from build123d import *

# Parameters (mm, degrees)
BOSS_EXTRUDE1_DEPTH = 9
SKETCH2_R           = 15
BOSS_EXTRUDE2_DEPTH = 4
SKETCH3_R           = 7.5
BOSS_EXTRUDE3_DEPTH = 2
SKETCH4_R           = 11
BOSS_EXTRUDE5_DEPTH = 13
CHAMFER1_SIZE       = 2
SCALE_1_SCALE       = 1.875


with BuildPart() as part:
    # Sketch1 → Boss-Extrude1 (new body)
    with BuildSketch(Plane.XY):
        Polygon((14.43375673, 0), (7.216878365, 12.5), (-7.216878365, 12.5), (-14.43375673, 0), (-7.216878365, -12.5), (7.216878365, -12.5), align=None)
    extrude(amount=BOSS_EXTRUDE1_DEPTH)

    # Sketch2 → Boss-Extrude2 (add)
    with BuildSketch(Plane.XY.offset(9)):
        Circle(SKETCH2_R)
    extrude(amount=BOSS_EXTRUDE2_DEPTH)

    # Sketch3 → Boss-Extrude3 (add)
    with BuildSketch(Plane.XY.offset(13)):
        Circle(SKETCH3_R)
    extrude(amount=BOSS_EXTRUDE3_DEPTH)

    # Sketch4 → Boss-Extrude5 (add)
    with BuildSketch(Plane.XY.offset(15)):
        with Locations(Location((0, 0, 0), (0, 0, 180))):
            Circle(SKETCH4_R)
    extrude(amount=BOSS_EXTRUDE5_DEPTH)

    # Chamfer1
    chamfer1_edges = [part.edges().sort_by_distance(p)[0] for p in [
        (11, 0, 28),
    ]]
    chamfer(chamfer1_edges, length=CHAMFER1_SIZE)

    # Sketch6 → Cut-Revolve4 (revolve, cut)
    with BuildSketch(Plane(origin=(0, 0, 0), x_dir=(1, 0, 0), z_dir=(0, 1, 0)), mode=Mode.PRIVATE) as cut_revolve4_sk:
        with BuildLine():
            Line((-10.43375673, 0), (-11.300713231, 3.45481125))
            Line((-11.300713231, 3.45481125), (-14.43375673, 0))
            Line((-14.43375673, 0), (-14.43375673, -1))
            ThreePointArc((-14.43375673, -1), (-12.499286844, -0.237879543), (-10.43375673, 0))
        make_face()
    revolve(cut_revolve4_sk.sketch.rotate(Axis((0, 0, 0), (0, 0, -1)), 180), axis=Axis((0, 0, 0), (0, 0, -1)), mode=Mode.SUBTRACT)


with BuildPart() as part_1:
    # Scale 1: scaled about (-3.1e-08, 2.41e-07, 12.521211358)
    add(part.part.scale(SCALE_1_SCALE).moved(Location((2.7e-08, -2.11e-07, -10.956059938))))


solid = part_1.part
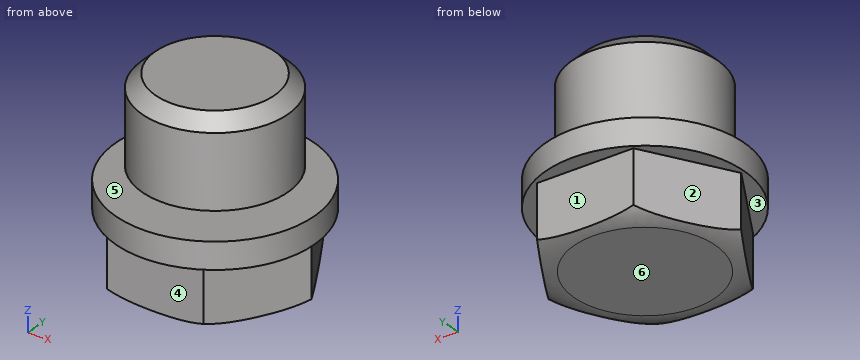
Design review of the part built by this model. Coordinates are the model's own, in mm. Face numbers are marked on the shaded views. A direction names the side the tool comes from. Round coordinates to 2 decimals unless told otherwise and drop trailing zeros. Write each loop counter-clockwise with the first axis right and the second up, starting at its lowest first coordinate (ties: lowest second). Pieces come first, ordered by that corner, then holes. Notation, with made-up numbers: M 35.25,-14 L 45.25,-14 A38 cw 45.25,25 Z; hole C 5,68.25 d4. An arc over 180 degrees is marked long. One line per item, written item: value. Start each with the question number.
1. To check wall thickness, follow probe 1 along Z at (x, y) = (13, -19.5); probe 2 along Y at (x, z) = (-9, -8.5); probe 3 along Z at (x, y) = (11, -13). State the ranges of each line that lie inside material, in increasing order. Write a range as from..to.
2. Draft analysis for pull direction Z (two halves, no side actions). For the marked faces 4, 5 and 6, state which applies: pulls with the +Z half, pulls with the -Z half, needs draft (parallel to the pull), parting line crosses it, or undercut.
3. Take a section at B-B on z = 25.5. State the section outline as (x, y) points (3 decimals).
4. Clearance check with flat-ended pins moving along their axes: P1, Ø8, axis at x = 6, z = 32.5, coming from the -Y side; P2, Ø13, axis at x = 5, z = -1.5, coming from the +Y side; P3, Ø1.5, axis at x = 0, z = 30, coming from the -Y side (3 decimals). State where each tip first meets the part, or that it passes through.
5. Take a section at C-C on z = 9.5. State the section outline as (x, y) points (3 decimals), then the cut area to 3 significant figures.
6. Take a section at A-A on z = 0.5. State the section outline as (x, y) points.
7. For the marked faces 1, 2 and 3, list the 3-axis set-ups (+Z, -Z, +X, -X, +Y, -Y) from which the entire face can be reached by the end or side of a thin tool; tool diameter is ignored.
Computed:
1. probe 1: z = -10.51..13.42
1. probe 2: y = -23.44..23.44
1. probe 3: z = -10.96..13.42, 17.17..41.39
2. face 4: needs draft
2. face 5: undercut
2. face 6: pulls with the -Z half
3. outline: C 0,0 d41.25
4. P1: stops at y = -20.53
4. P2: stops at y = 23.44
4. P3: stops at y = -20.625
5. outline: C 0,0 d56.25
5. area: 2,490 mm²
6. outline: M -27.06,0 L -13.53,-23.44 L 13.53,-23.44 L 27.06,0 L 13.53,23.44 L -13.53,23.44 Z
7. face 1: -Z, +X, -X, +Y
7. face 2: -Z, -X, +Y
7. face 3: -Z
